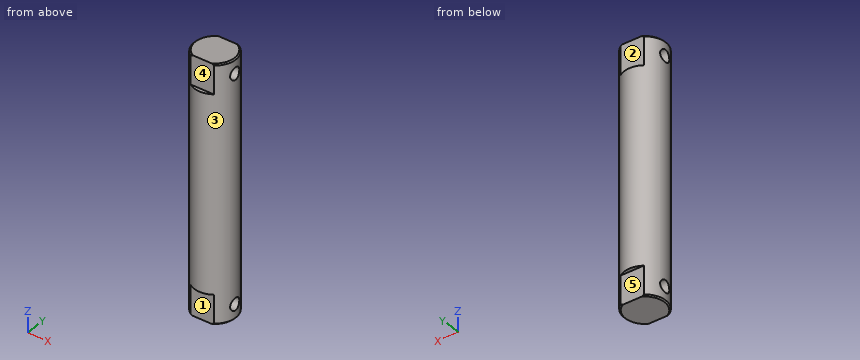
from build123d import *

# Parameters (mm, degrees)
SKETCH_1_R          = 8.5
EXTRUDE_1_DEPTH     = 52
SKETCH_2_W          = 25
SKETCH_2_H          = 3
CUT_EXTRUDE_1_DEPTH = 12
CHAMFER_2_SIZE      = 0.5
HOLE_WIZARD_M6_1_D  = 5


with BuildPart() as part:
    # 草图1 → 凸台-拉伸1 (new, symmetric)
    with BuildSketch(Plane.XY):
        with Locations(Location((0, 0, 0), (0, 0, 180))):
            Circle(SKETCH_1_R)
    extrude(amount=EXTRUDE_1_DEPTH, both=True)

    # 草图2 → 切除-拉伸1 (cut)
    with BuildSketch(Plane.XY.offset(52)):
        with Locations((0, 8.5)):
            Rectangle(SKETCH_2_W, SKETCH_2_H)
        with Locations((0, -8.5)):
            Rectangle(SKETCH_2_W, SKETCH_2_H)
    cut_extrude_1 = extrude(amount=-CUT_EXTRUDE_1_DEPTH, mode=Mode.SUBTRACT)

    # 镜向1: 切除-拉伸1 across plane
    add(cut_extrude_1.mirror(Plane.XY), mode=Mode.SUBTRACT)

    # 倒角2
    chamfer_2_edges = [part.edges().sort_by_distance(p)[0] for p in [
        (8.5, 0, 52),
        (-7.524477249, 3.953763034, -52),
        (8.5, 0, -52),
        (-7.524477249, 3.953763034, 52),
    ]]
    chamfer(chamfer_2_edges, length=CHAMFER_2_SIZE)

    # M6 螺纹孔1 (through all)
    with Locations(Plane(origin=(8.5, 0, 0), x_dir=(0, 0, -1), z_dir=(1, 0, 0))):
        with Locations((-46, 0), (46, 0)):
            Hole(HOLE_WIZARD_M6_1_D / 2)


solid = part.part
Work out the finished part from the listing and answer in its coordinate system (mm). Face numbers are marked on the shaded views. A direction names the side the tool comes from. Round coordinates to 2 decimals unless told otherwise and drop trailing zeros. Loops run counter-clockwise (first coordinate to the right, second up) from the corner with the lowest first, then second, coordinate; pieces in that order, holes last. Notation, with made-up numbers: (64, 13.25) - (76, 13.25) arc R19 ccw to (76, 27.25) - close; hole circle Ø7 at (87.5, 57). An arc over 180 degrees is marked (long way). Use one line per item in the form item = value. Start each with the question number.
(1) Which of the six approach directions +Z, -Z, +X, -X, +Y, -Y give full straight-line access (tool end or side, diameter ignored) to the marked faces 1, 2, 3, 4 and 5?
(2) Find section C-C on z = -46. Determine the outline of the cut face in (x, y).
(3) Find section A-A on y = 0. Determine the outline of the cut face in (x, z), and give its area (3 significant figures).
(4) Flat-ended cylindrical pins translate along their axes: P1, Ø6, axis at y = -4, z = -32, coming from the -X side; P2, Ø7.5, axis at x = 1.5, z = -43.5, coming from the -Y side; P3, Ø0.8, axis at x = -1.5, y = 8, coming from the +Z side; P4, Ø3, axis at y = 0, z = -46, coming from the -X side. Find the tip coordinate at first contact, or state that the pin passes through.
(5) Consider line 1 (Z direction, x = -3.75, y = 0); line 2 (Y direction, x = -3.5, z = -46); line 3 (Z direction, x = -6.5, y = 2.25). Determine where each line is inside the solid, lowest interval first.
(6) Find section B-B on x = 0. Determine the outline of the cut face in (y, z).
(7) Find section D-D on z = 4.5. Determine the outline of the cut face in (x, y).
Answer list:
q1.face_1 = -Z, +X, -X, -Y
q1.face_2 = +Z, +X, -X, +Y
q1.face_3 = +Z, -Z
q1.face_4 = +Z, +X, -X, -Y
q1.face_5 = -Z, +X, -X, +Y
q2.outline = (-8.12, -2.5) arc R8.5 ccw to (-4.82, -7) - (4.82, -7) arc R8.5 ccw to (8.12, -2.5) - close; (-8.12, 2.5) - (8.12, 2.5) arc R8.5 ccw to (4.82, 7) - (-4.82, 7) arc R8.5 ccw to start
q3.outline = (-8.5, -51.5) - (-8, -52) - (8, -52) - (8.5, -51.5) - (8.5, -48.5) - (-8.5, -48.5) - close; (-8.5, -43.5) - (8.5, -43.5) - (8.5, 43.5) - (-8.5, 43.5) - close; (-8.5, 48.5) - (8.5, 48.5) - (8.5, 51.5) - (8, 52) - (-8, 52) - (-8.5, 51.5) - close
q3.area = 1,600 mm^2
q4.P1 = -8.44
q4.P2 = -8.5
q4.P3 = 40
q4.P4 = through
q5.line_1 = -52 to -48.5, -43.5 to 43.5, 48.5 to 52
q5.line_2 = -7 to -2.5, 2.5 to 7
q5.line_3 = -52 to -47.09, -44.91 to 44.91, 47.09 to 52
q6.outline = (-8.5, -40) - (-7, -40) - (-7, -52) - (7, -52) - (7, -40) - (8.5, -40) - (8.5, 40) - (7, 40) - (7, 52) - (-7, 52) - (-7, 40) - (-8.5, 40) - close; hole circle Ø5 at (0, -46); hole circle Ø5 at (0, 46)
q7.outline = circle Ø17 at (0, 0)
